Design review of the part built by this model. Coordinates are the model's own, in mm. Round coordinates to 2 decimals unless told otherwise and drop trailing zeros. Write each loop counter-clockwise with the first axis right and the second up, starting at its lowest first coordinate (ties: lowest second). Pieces come first, ordered by that corner, then holes. Notation, with made-up numbers: M 65,74.5 L 91,74.5 A22 ccw 91,85.5 Z; hole C 85.25,12 d9. An arc over 180 degrees is marked long. Use CSV: the item, a comma, the result in double quotes.
from build123d import *

# Parameters (mm, degrees)
EXTRUDE1_DEPTH = 5
SKETCH2_R      = 4
EXTRUDE2_DEPTH = 10


with BuildPart() as part:
    # Sketch1 → Extrude1 (new, symmetric)
    with BuildSketch(Plane.XY):
        Polygon((-80, 0), (0, 0), (0, -300), (-20, -300), align=None)
    extrude(amount=EXTRUDE1_DEPTH, both=True)

    # Sketch2 → Extrude2 (cut)
    with BuildSketch(Plane.XY.offset(5)):
        with Locations((-25, -160)):
            Circle(SKETCH2_R)
        with Locations((-25, -181)):
            Circle(SKETCH2_R)
    extrude(amount=-EXTRUDE2_DEPTH, mode=Mode.SUBTRACT)


solid = part.part
1) Add section C-C on z = 1.75. Write out the cut boundary in (x, y), then the cut area to 3 significant figures.
Answers:
outline,"M -80,0 L -20,-300 L 0,-300 L 0,0 Z; hole C -25,-181 d8; hole C -25,-160 d8"
area,"14,900 mm²"
2) The part is to be moulded in two halves that separate along Y. For faces 1 (the face through (-25.521, -156.034, 0.07)), 2 (the face through (0, -148, 0)), 3 (the face through (-10, -300, 0)), say which applies: released by +Y, released by -Y, zero draft, split by the parting line, or undercut.
Answers:
face 1,"undercut"
face 2,"zero draft"
face 3,"released by -Y"
3) Add section D-D on x = -56.5. Write out the cut boundary in (y, z).
Answers:
outline,"M -117.5,-5 L 0,-5 L 0,5 L -117.5,5 Z"
4) For pin 1 Ø4 at (y, z) = (-90, -4) entering from -X, flat-tipped, find the tip position at first contact; note if it passes through.
Answers:
pin 1,"x = -62.4"
5) Add section A-A on x = -25. Write out the cut boundary in (y, z).
Answers:
outline,"M -275,-5 L -185,-5 L -185,5 L -275,5 Z; M -177,-5 L -164,-5 L -164,5 L -177,5 Z; M -156,-5 L 0,-5 L 0,5 L -156,5 Z"
6) Wall thickness on line 1 along X through (y, z) = (-196, -3); line 2 along X through (y, z) = (-18, -0.5): over which ranges is each line inside the solid? List them lowest first. Write a range as [from, to].
Answers:
line 1,"[-40.8, 0]"
line 2,"[-76.4, 0]"
7) Add section B-B on y = -160. Write out the cut boundary in (x, z).
Answers:
outline,"M -48,-5 L -29,-5 L -29,5 L -48,5 Z; M -21,-5 L 0,-5 L 0,5 L -21,5 Z"
